```python
from build123d import *

# Parameters (mm, degrees)
EXTRUDE_1_DEPTH              = 60
SKETCH_3_W                   = 50
SKETCH_3_H                   = 15.1
CUT_EXTRUDE_1_DEPTH          = 2
HOLE_WIZARD_M4_1_D           = 4.5
HOLE_WIZARD_M4_1_CBORE_D     = 8
HOLE_WIZARD_M4_1_CBORE_DEPTH = 4.4
HOLE_WIZARD_M6_1_D           = 6.6
HOLE_WIZARD_M6_1_CBORE_D     = 11
HOLE_WIZARD_M6_1_CBORE_DEPTH = 6.4
HOLE_WIZARD_M6_2_D           = 6.6
HOLE_WIZARD_M6_2_CBORE_D     = 11
HOLE_WIZARD_M6_2_CBORE_DEPTH = 6.4
CHAMFER_1_SIZE               = 2
HOLE_WIZARD_M6_1_2_D         = 5
HOLE_WIZARD_M6_1_2_DEPTH     = 17
HOLE_WIZARD_M6_1_2_TIP       = 1.502151548


with BuildPart() as part:
    # 草图2 → 凸台-拉伸1 (new body)
    with BuildSketch(Plane.XY):
        Polygon((50, 0), (0, 0), (0, 30), (10, 30), (10, 10), (50, 10), align=None)
    extrude(amount=EXTRUDE_1_DEPTH)

    # 草图3 → 切除-拉伸1 (cut)
    with BuildSketch(Plane.XZ):
        with Locations((25, 12.55)):
            Rectangle(SKETCH_3_W, SKETCH_3_H)
    extrude(amount=-CUT_EXTRUDE_1_DEPTH, mode=Mode.SUBTRACT)

    # M4 六角凹头螺钉的柱形沉头孔1 (through all)
    with Locations(Plane(origin=(0, 30, 0), x_dir=(1, 0, 0), z_dir=(0, 1, 0))):
        with Locations((5, -12.55)):
            CounterBoreHole(HOLE_WIZARD_M4_1_D / 2, HOLE_WIZARD_M4_1_CBORE_D / 2, HOLE_WIZARD_M4_1_CBORE_DEPTH)

    # Hole Wizard M6 _1 (through all)
    with Locations(Plane(origin=(0, 10, 0), x_dir=(1, 0, 0), z_dir=(0, 1, 0))):
        with Locations((20, -12.55), (40, -12.55)):
            CounterBoreHole(HOLE_WIZARD_M6_1_D / 2, HOLE_WIZARD_M6_1_CBORE_D / 2, HOLE_WIZARD_M6_1_CBORE_DEPTH)

    # M6 六角凹头螺钉的柱形沉头孔2 (through all)
    with Locations(Plane.ZY):
        with Locations((30.05, 20), (50.05, 20)):
            CounterBoreHole(HOLE_WIZARD_M6_2_D / 2, HOLE_WIZARD_M6_2_CBORE_D / 2, HOLE_WIZARD_M6_2_CBORE_DEPTH)

    # 倒角1
    chamfer_1_edges = [part.edges().sort_by_distance(p)[0] for p in [
        (5, 30, 60),
        (50, 5, 60),
        (5, 30, 0),
        (50, 5, 0),
    ]]
    chamfer(chamfer_1_edges, length=CHAMFER_1_SIZE)

    # Hole Wizard M6 _1 2
    with Locations(Plane(origin=(0, 0, 0), x_dir=(-1, 0, 0), z_dir=(0, -1, 0))):
        with Locations((-37.5, -45.1), (-12.5, -45.1)):
            Hole(HOLE_WIZARD_M6_1_2_D / 2, depth=HOLE_WIZARD_M6_1_2_DEPTH)
            with Locations((0, 0, -(HOLE_WIZARD_M6_1_2_DEPTH + HOLE_WIZARD_M6_1_2_TIP / 2))):  # 118° drill point
                Cone(0, HOLE_WIZARD_M6_1_2_D / 2, HOLE_WIZARD_M6_1_2_TIP, mode=Mode.SUBTRACT)


solid = part.part
```
Read the model definition and answer for the solid it produces. Units are mm, in the model's axes. A direction names the side the tool comes from. Round coordinates to 2 decimals unless told otherwise and drop trailing zeros. Write each loop counter-clockwise with the first axis right and the second up, starting at its lowest first coordinate (ties: lowest second). Pieces come first, ordered by that corner, then holes. Notation, with made-up numbers: (-8.75, 83) - (11.25, 83) arc R19 cw to (11.25, 104) - close; hole circle Ø7 at (89.5, 79.25). An arc over 180 degrees is marked (long way). One line per item, written item: value.
Q1. Which of the six approach directions +Z, -Z, +X, -X, +Y, -Y give full straight-line access (tool end or side, diameter ignored) to faces 5 (the cylindrical face through (10.66, 5.07, 43.41)), 6 (the flat face through (6.4, 16, 30)), 7 (the cylindrical face through (34.505, 6.845, 12.308)), 8 (the flat face through (25, 1, 20.1))?
The answers:
face 5: +Y, -Y
face 6: -X
face 7: +Y
face 8: +X, -X, -Y
Q2. Find section A-A (y = 20). Determine the outline of the cut face in (x, z).
The answers:
outline: (0, 0) - (10, 0) - (10, 26.75) - (6.4, 26.75) - (6.4, 24.55) - (0, 24.55) - close; (0, 35.55) - (6.4, 35.55) - (6.4, 33.35) - (10, 33.35) - (10, 46.75) - (6.4, 46.75) - (6.4, 44.55) - (0, 44.55) - close; (0, 55.55) - (6.4, 55.55) - (6.4, 53.35) - (10, 53.35) - (10, 60) - (0, 60) - close; hole circle Ø4.5 at (5, 12.55)
Q3. Find section C-C (z = 50.05). Determine the outline of the cut face in (x, y), and give its area (3 significant figures).
The answers:
outline: (0, 0) - (50, 0) - (50, 10) - (10, 10) - (10, 16.7) - (6.4, 16.7) - (6.4, 14.5) - (0, 14.5) - close; (0, 25.5) - (6.4, 25.5) - (6.4, 23.3) - (10, 23.3) - (10, 30) - (0, 30) - close
area: 606 mm2
Q4. Each of these flat-tipped pins is pushed along its axis until it touches: P1, Ø5, axis at y = 19, z = 49, coming from the -X side; P2, Ø6.5, axis at x = 40, z = 12.55, coming from the +Y side; P3, Ø1, axis at y = 25, z = 9.5, coming from the -X side; P4, Ø1.5, axis at y = 25.5, z = 28, coming from the +X side. Where does it stop, or does it pass through?
The answers:
P1: stops at x = 6.4
P2: passes through
P3: stops at x = 0
P4: stops at x = 10
Q5. Find section D-D (y = 5.75). Determine the outline of the cut face in (x, z), and give its area (3 significant figures).
The answers:
outline: (0, 0) - (48, 0) - (50, 2) - (50, 58) - (48, 60) - (0, 60) - close; hole circle Ø4.5 at (5, 12.55); hole circle Ø5 at (12.5, 45.1); hole circle Ø11 at (20, 12.55); hole circle Ø11 at (40, 12.55); hole circle Ø5 at (37.5, 45.1)
area: 2,750 mm2
Q6. Find section B-B (x = 12.5). Determine the outline of the cut face in (y, z).
The answers:
outline: (0, 0) - (10, 0) - (10, 42.6) - (0, 42.6) - (0, 20.1) - (2, 20.1) - (2, 5) - (0, 5) - close; (0, 47.6) - (10, 47.6) - (10, 60) - (0, 60) - close
Q7. For a pull along X with two mould halves and no side action, classify faces 1 (the flat face through (19.9, 3.6, 16.1)), 2 (the cylindrical face through (8.225, 20.145, 33.347)), 3 (the cylindrical face through (16.95, 2.79, 13.81)), 4 (the flat face through (0, 11, 30)) as pulls with the +X half, pulls with the -X half, needs draft (parallel to the pull), parting line crosses it, or undercut.
The answers:
face 1: undercut
face 2: needs draft
face 3: undercut
face 4: pulls with the -X half
Q8. Straight lines are drawn through the part: line 1 (X direction, y = 2.5, z = 45.1); line 2 (X direction, y = 2.7, z = 12.55); line 3 (Y direction, x = 42, z = 54). For each, find the intervals that lie inside material, in ascending order. Write a range as from..to.
The answers:
line 1: x = 0..10, 15..35, 40..50
line 2: x = 0..2.75, 7.25..16.7, 23.3..36.7, 43.3..50
line 3: y = 0..10
